Drawing for the job (mm, zero at the part's lowest x, y, z). Coordinates: 2 decimals unless noted, no trailing zeros. Order: outer loops, then holes, each group sorted by start corner. A loop starts at its lowest first (then second) coordinate and runs counter-clockwise, first axis right, second up.
1) Wall check: L1, parallel to X at y = 12, z = 22.5; L2, parallel to Z at x = 20, y = 11.75; L3, parallel to Z at x = 73.5, y = 5.5. Give the ranges that are in metal, low to high.
2) Cut at C-C (y = 2.5). List the corners of the cut face in (x, z), and give its area (3 significant figures).
3) Cut at A-A (z = 99.5). List the corners of the cut face in (x, y), and give its area (3 significant figures).
4) Cut at B-B (x = 20). List the corners of the cut face in (y, z), and give its area (3 significant figures).
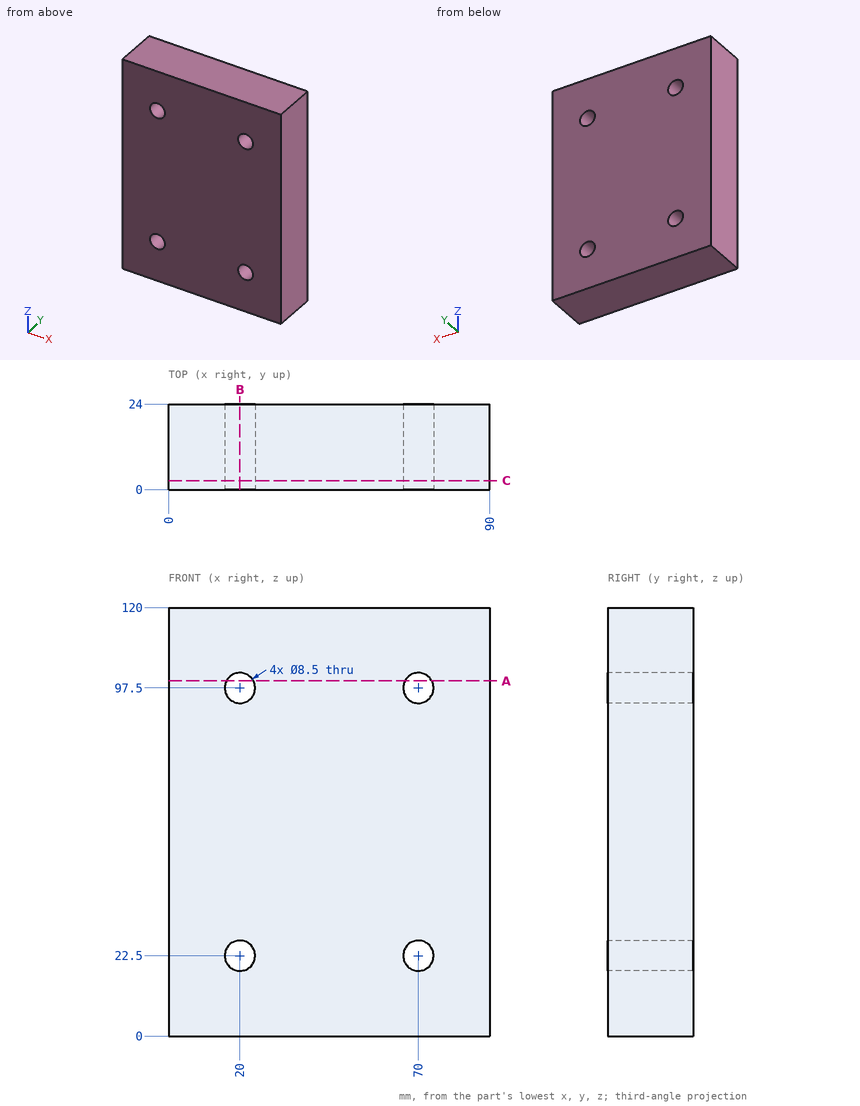
Geometry check:
1. L1: x = 0 to 15.75, 24.25 to 65.75, 74.25 to 90
1. L2: z = 0 to 18.25, 26.75 to 93.25, 101.75 to 120
1. L3: z = 0 to 20.09, 24.91 to 95.09, 99.91 to 120
2. outline: (0, 0) - (90, 0) - (90, 120) - (0, 120) - close; hole circle Ø8.5 at (20, 22.5); hole circle Ø8.5 at (20, 97.5); hole circle Ø8.5 at (70, 22.5); hole circle Ø8.5 at (70, 97.5)
2. area: 10,600 mm2
3. outline: (0, 0) - (16.25, 0) - (16.25, 24) - (0, 24) - close; (23.75, 0) - (66.25, 0) - (66.25, 24) - (23.75, 24) - close; (73.75, 0) - (90, 0) - (90, 24) - (73.75, 24) - close
3. area: 1,800 mm2
4. outline: (0, 0) - (24, 0) - (24, 18.25) - (0, 18.25) - close; (0, 26.75) - (24, 26.75) - (24, 93.25) - (0, 93.25) - close; (0, 101.75) - (24, 101.75) - (24, 120) - (0, 120) - close
4. area: 2,470 mm2
